from build123d import *

# Parameters (mm, degrees)
BASE_PLATE_SKETCH_W         = 115
BASE_PLATE_SKETCH_H         = 210
BASE_PLATE_115X210X30_DEPTH = 15
UPRIGHT_PROFILE_SKETCH_R    = 8.394069109
UPRIGHT_PROFILE_SKETCH_R_2  = 9.244434853
UPRIGHT_BODY_DEPTH          = 50
UPRIGHT_ROUND_RADIUS        = 57.5
UPRIGHT_ROUND_LENGTH        = 100
SADDLE_CUT_DEPTH            = 75
SIDE_BOSS_SKETCH_W          = 8
SIDE_BOSS_SKETCH_H          = 45
SIDE_BOSS_DEPTH             = 57.5
EDGE_FILLET_R20_R           = 20


with BuildPart() as part:
    # Base Plate Sketch → Base Plate 115x210x30 (new, symmetric)
    with BuildSketch(Plane(origin=(0, 0, 0), x_dir=(1, 0, 0), z_dir=(0, 1, 0))):
        Rectangle(BASE_PLATE_SKETCH_W, BASE_PLATE_SKETCH_H)
    extrude(amount=BASE_PLATE_115X210X30_DEPTH, both=True)

    # Upright Profile Sketch → Upright Body (add, symmetric)
    with BuildSketch(Plane.XY):
        with BuildLine():
            Line((57.5, 47), (35, 47))
            ThreePointArc((35, 47), (31.464466094, 45.535533906), (30, 42))
            Line((30, 42), (30, 15))
            Line((30, 15), (-30, 15))
            Line((-30, 15), (-30, 42))
            ThreePointArc((-30, 42), (-31.464466094, 45.535533906), (-35, 47))
            Line((-35, 47), (-57.5, 47))
            Line((-57.5, 47), (-57.5, 258))
            Line((-57.5, 258), (57.5, 258))
            Line((57.5, 258), (57.5, 47))
        make_face()
        with Locations((0, 220.5)):
            Circle(UPRIGHT_PROFILE_SKETCH_R, mode=Mode.SUBTRACT)
        with Locations((0, 78.5)):
            Circle(UPRIGHT_PROFILE_SKETCH_R_2, mode=Mode.SUBTRACT)
    extrude(amount=UPRIGHT_BODY_DEPTH, both=True)

    # Upright Round: full round fillet: the end face becomes a half cylinder, R = half its width
    upright_round_face = Plane((0, 258, 0), x_dir=(0, 0, 1), z_dir=(0, 1, 0))  # on the end face: x along it, z out of the body
    upright_round_slab = upright_round_face.offset(-UPRIGHT_ROUND_RADIUS / 2) * Box(UPRIGHT_ROUND_LENGTH, 2 * UPRIGHT_ROUND_RADIUS, UPRIGHT_ROUND_RADIUS, mode=Mode.PRIVATE)  # the body's end, R deep
    upright_round_round = Plane((0, 200.5, 0), x_dir=(0, 1, 0), z_dir=(0, 0, 1)) * Cylinder(UPRIGHT_ROUND_RADIUS, UPRIGHT_ROUND_LENGTH, mode=Mode.PRIVATE)  # its axis R under the face
    add(upright_round_slab - upright_round_round, mode=Mode.SUBTRACT)

    # Saddle Cut Sketch → Saddle Cut (cut, symmetric)
    with BuildSketch(Plane(origin=(0, 0, 0), x_dir=(0, 0, -1), z_dir=(1, 0, 0))):
        with BuildLine():
            Line((-50, 183), (10, 183))
            ThreePointArc((10, 183), (50, 143), (10, 103))
            Line((10, 103), (-50, 103))
            Line((-50, 103), (-50, 183))
        make_face()
    extrude(amount=SADDLE_CUT_DEPTH, both=True, mode=Mode.SUBTRACT)


with BuildPart() as saddle_cut_piece_1:
    # of the separate pieces the step leaves, piece 1, a body of its own (saddle_cut_pieces)
    add(part.part.solids().sort_by_distance((-57.5, -15, -105))[0])



with BuildPart() as saddle_cut_piece_2:
    # of the separate pieces the step leaves, piece 2, a body of its own (saddle_cut_pieces)
    add(part.part.solids().sort_by_distance((-57.5, 200.5, -50))[0])


with BuildPart() as saddle_cut_piece_1_1:
    add(saddle_cut_piece_1.part)

    add(saddle_cut_piece_2.part)  # Side Boss merges Saddle Cut piece 2
    # Side Boss Sketch → Side Boss (add, symmetric)
    with BuildSketch(Plane(origin=(0, 0, 0), x_dir=(0, 0, -1), z_dir=(1, 0, 0))):
        with Locations((54, 143)):
            Rectangle(SIDE_BOSS_SKETCH_W, SIDE_BOSS_SKETCH_H)
    extrude(amount=SIDE_BOSS_DEPTH, both=True)

    # Edge Fillet R20
    edge_fillet_r20_edges = [saddle_cut_piece_1_1.edges().sort_by_distance(p)[0] for p in [
        (0, 15, 50),
        (0, 15, -50),
    ]]
    fillet(edge_fillet_r20_edges, radius=EDGE_FILLET_R20_R)


solid = saddle_cut_piece_1_1.part
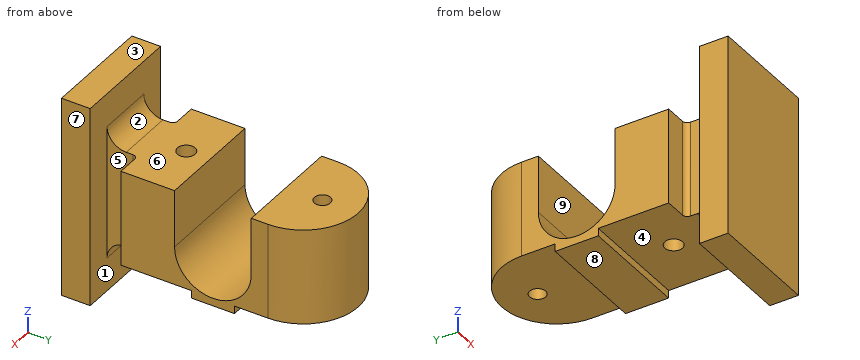
Verification items for the finished model (mm, model axes). Face numbers are marked on the shaded views. A direction names the side the tool comes from. Coordinates: 2 decimals unless noted, no trailing zeros. Write each loop counter-clockwise with the first axis right and the second up, starting at its lowest first coordinate (ties: lowest second). Pieces come first, ordered by that corner, then holes. Notation, with made-up numbers: M -33.5,71 L -10.5,71 A28 ccw -10.5,96 Z; hole C -0.5,51 d5. An arc over 180 degrees is marked long. Use CSV: the item, a comma, the result in double quotes.
Q1. Mould release check, pull along Y, two halves, no side actions. Record for the marked faces 1, 2, 3 and 4: pulls with the +Y half, pulls with the -Y half, needs draft (parallel to the pull), parting line crosses it, or undercut.
Computed values:
face 1,"undercut"
face 2,"pulls with the +Y half"
face 3,"needs draft"
face 4,"undercut"
Q2. Thickness scan on line 1 along Y through (x, z) = (0, -1); line 2 along Y through (x, z) = (-5.5, 31); line 3 along Y through (x, z) = (8.5, 3.5). Record the ranges inside material, lowest first. Write a range as [from, to].
Computed values:
line 1,"[-15, 69.26], [87.74, 103], [183, 212.11], [228.89, 258]"
line 2,"[-15, 71.07], [85.93, 103], [183, 214.16], [226.84, 257.74]"
line 3,"[-15, 74.87], [82.13, 103], [183, 257.37]"
Q3. Set-up check for the marked faces 5, 6, 7, 8 and 9: record each of +Z, -Z, +X, -X, +Y, -Y from which the full face is reachable in a straight line by a thin tool's end or side.
Computed values:
face 5,"+Z, -Z, +X"
face 6,"+Z, +X, -X, +Y"
face 7,"+Z, -Z, +X, +Y, -Y"
face 8,"-Z, +X, -X, +Y"
face 9,"+Z, +X, -X"
Q4. Section check B-B, the plane y = 78.5. Enter the section's corners in (x, z).
Computed values:
outline,"M -57.5,-50 L -9.24,-50 L -9.24,50 L -57.5,50 Z; M 9.24,-50 L 57.5,-50 L 57.5,50 L 9.24,50 Z"
Q5. Section check C-C, the plane x = 48. Enter the section's corners in (y, z), and give its area (3 significant figures).
Computed values:
outline,"M -15,-105 L 15,-105 L 15,105 L -15,105 Z; M 47,-50 L 120.5,-50 L 120.5,-58 L 165.5,-58 L 165.5,-50 L 232.16,-50 L 232.16,50 L 183,50 L 183,-10 A40 cw 103,-10 L 103,50 L 47,50 Z"
area,"17,900 mm²"
Q6. Go/stop test with flat-tipped pins: P1, Ø13.5, axis at x = 15, y = 143.5, coming from the -Z side; P2, Ø1.5, axis at y = 22, z = -46.5, coming from the -X side; P3, Ø1.5, axis at x = 27.5, z = -50, coming from the +Y side; P4, Ø10, axis at x = 0, y = 220.5, coming from the -Z side. Record where each tip stops, or that it passes through.
Computed values:
P1,"z = -58"
P2,"x = -30"
P3,"y = 251.4"
P4,"through"
Q7. Section check A-A, the plane z = 47. Enter the section's corners in (x, y), and give its area (3 significant figures).
Computed values:
outline,"M -57.5,-15 L 57.5,-15 L 57.5,15 L 30,15 L 30,42 A5 cw 35,47 L 57.5,47 L 57.5,103 L -57.5,103 L -57.5,47 L -35,47 A5 cw -30,42 L -30,15 L -57.5,15 Z; M -57.5,183 L 57.5,183 L 57.5,200.5 A57.5 ccw -57.5,200.5 Z; hole C 0,78.5 d18.49; hole C 0,220.5 d16.79"
area,"18,500 mm²"
Q8. Section check D-D, the plane y = 220.5. Enter the section's corners in (x, z).
Computed values:
outline,"M -53.91,-50 L -8.39,-50 L -8.39,50 L -53.91,50 Z; M 8.39,-50 L 53.91,-50 L 53.91,50 L 8.39,50 Z"
